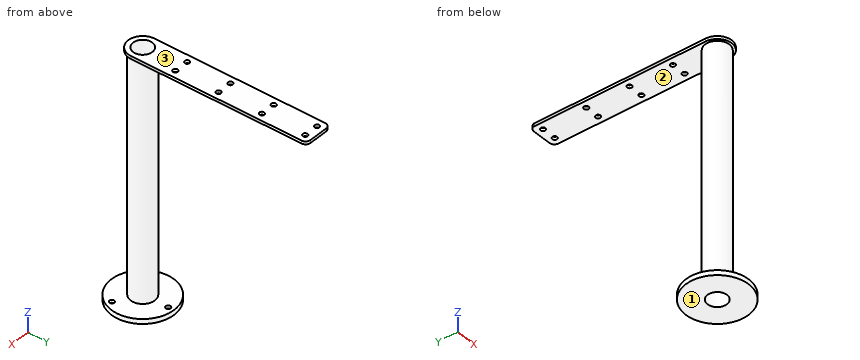
from build123d import *

# Parameters (mm, degrees)
SKETCH1_R           = 65
SKETCH1_R_2         = 20
BOSS_EXTRUDE1_DEPTH = 10
SKETCH2_R           = 25
SKETCH2_R_2         = 20
BOSS_EXTRUDE2_DEPTH = 494
SKETCH3_R           = 20
BOSS_EXTRUDE3_DEPTH = 6
FILLET1_R           = 10
SKETCH4_R           = 5
CUT_EXTRUDE1_DEPTH  = 6
SKETCH5_R           = 5
CUT_EXTRUDE2_DEPTH  = 6


with BuildPart() as part:
    # Sketch1 → Boss-Extrude1 (new body)
    with BuildSketch(Plane.XY):
        Circle(SKETCH1_R)
        Circle(SKETCH1_R_2, mode=Mode.SUBTRACT)
    extrude(amount=BOSS_EXTRUDE1_DEPTH)

    # Sketch2 → Boss-Extrude2 (add)
    with BuildSketch(Plane.XY.offset(10)):
        Circle(SKETCH2_R)
        Circle(SKETCH2_R_2, mode=Mode.SUBTRACT)
    extrude(amount=BOSS_EXTRUDE2_DEPTH)

    # Sketch3 → Boss-Extrude3 (add)
    with BuildSketch(Plane.XY.offset(504)):
        with BuildLine():
            Line((-30, 0), (-30, 365))
            Line((-30, 365), (30, 365))
            Line((30, 365), (30, 0))
            ThreePointArc((30, 0), (0, -30), (-30, 0))
        make_face()
        Circle(SKETCH3_R, mode=Mode.SUBTRACT)
    extrude(amount=BOSS_EXTRUDE3_DEPTH)

    # Fillet1
    fillet1_edges = [part.edges().sort_by_distance(p)[0] for p in [
        (30, 365, 507),
        (-30, 365, 507),
    ]]
    fillet(fillet1_edges, radius=FILLET1_R)

    # Sketch4 → Cut-Extrude1 (cut)
    with BuildSketch(Plane.XY.offset(510)):
        with Locations((-15, 350)):
            Circle(SKETCH4_R)
        with Locations((15, 350)):
            Circle(SKETCH4_R)
        with Locations((-15, 260)):
            Circle(SKETCH4_R)
        with Locations((15, 260)):
            Circle(SKETCH4_R)
        with Locations((-15, 170)):
            Circle(SKETCH4_R)
        with Locations((15, 170)):
            Circle(SKETCH4_R)
        with Locations((-15, 80)):
            Circle(SKETCH4_R)
        with Locations((15, 80)):
            Circle(SKETCH4_R)
    extrude(amount=-CUT_EXTRUDE1_DEPTH, mode=Mode.SUBTRACT)

    # Sketch5 → Cut-Extrude2 (cut)
    with BuildSketch(Plane.XY.offset(10)):
        with Locations((0, 53)):
            Circle(SKETCH5_R)
        with Locations((45.899346401, -26.5)):
            Circle(SKETCH5_R)
        with Locations((-45.899346401, -26.5)):
            Circle(SKETCH5_R)
    extrude(amount=-CUT_EXTRUDE2_DEPTH, mode=Mode.SUBTRACT)


solid = part.part
Design review of the part built by this model. Coordinates are the model's own, in mm. Face numbers are marked on the shaded views. Round coordinates to 2 decimals unless told otherwise and drop trailing zeros. Write each loop counter-clockwise with the first axis right and the second up, starting at its lowest first coordinate (ties: lowest second). Pieces come first, ordered by that corner, then holes. Notation, with made-up numbers: (-39.5, -30.75) -> (19.5, -30.75) arc R35 ccw to (19.5, 5.25) -> close; hole circle Ø4 at (-8.5, 81.25). An arc over 180 degrees is marked (long way). One line per item, written item: value. Start each with the question number.
Q1. Add section A-A (z = 175). Give the boundary of the cut face in (x, y).
Q2. Insertion check: P1, Ø13, axis at x = 15, y = 350, coming from the -Z side; P2, Ø6.5, axis at y = 172, z = 505.5, coming from the -X side; P3, Ø1.5, axis at y = 2, z = 192.5, coming from the +X side. Each pin has a flat end and moves straight along its axis. Give the tip position at first contact, or say it passes through.
Q3. Add section B-B (y = 131). Give the boundary of the cut face in (x, z).
Q4. To check wall thickness, follow probe 1 along X at (y, z) = (260, 505.9); probe 2 along Y at (x, z) = (0, 5); probe 3 along Y at (x, z) = (0, 361). State the ranges of each line that lie inside material, in increasing order.
Q5. The part is to be moulded in two halves that separate along Z. For the marked faces 1, 2 and 3, say which applies: pulls with the +Z half, pulls with the -Z half, needs draft (parallel to the pull), parting line crosses it, or undercut.
Response:
1. outline: circle Ø50 at (0, 0); hole circle Ø40 at (0, 0)
2. P1: stops at z = 504
2. P2: stops at x = -30
2. P3: stops at x = 24.97
3. outline: (-30, 504) -> (30, 504) -> (30, 510) -> (-30, 510) -> close
4. probe 1: x = -30 to -20, -10 to 10, 20 to 30
4. probe 2: y = -65 to -20, 20 to 48, 58 to 65
4. probe 3: y = -25 to -20, 20 to 25
5. face 1: pulls with the -Z half
5. face 2: undercut
5. face 3: pulls with the +Z half
